The model under review builds one solid part; all positions refer to its coordinate system, in mm. Face numbers are marked on the shaded views. Coordinates: 2 decimals unless noted, no trailing zeros. Loops run counter-clockwise (first coordinate to the right, second up) from the corner with the lowest first, then second, coordinate; pieces in that order, holes last. Notation, with made-up numbers: (41.5, 21.25) - (54.5, 21.25) arc R27 cw to (54.5, 44.25) - close; hole circle Ø5 at (5.5, 55). An arc over 180 degrees is marked (long way). One line per item, written item: value. Start each with the question number.
1. We need section B-B, the plane z = -6.5. Give the boundary of the cut face in (x, y), then the cut area to 3 significant figures.
2. We need section C-C, the plane x = 20. Give the boundary of the cut face in (y, z), then the cut area to 3 significant figures.
3. To check wall thickness, follow line 1 (X direction, y = 4.25, z = 16); line 2 (X direction, y = 9.1, z = 20); line 3 (Y direction, x = -10, z = -3). State the ranges of each line that lie inside material, in increasing order.
4. We need section A-A, the plane x = 0. Give the boundary of the cut face in (y, z), then the cut area to 3 significant figures.
5. Insertion check: P1, Ø3.5, axis at x = 16.5, z = -15.5, coming from the -Y side; P2, Ø1.8, axis at x = -16, z = 16, coming from the -Y side; P3, Ø14, axis at x = -2.5, z = -9.5, coming from the +Y side. Each pin has a flat end and moves straight along its axis. Give the tip position at first contact, or say it passes through.
6. We need section D-D, the plane z = 20. Give the boundary of the cut face in (x, y), then the cut area to 3 significant figures.
7. Mouldability with a two-part tool opening along Z and no side actions: class the marked faces 1, 2 and 3 as +Z half, -Z half, draft (parallel to the pull), parting line (faces both ways), or undercut.
from build123d import *

# Parameters (mm, degrees)
SKETCH1_W           = 50
SKETCH1_H           = 50
BOSS_EXTRUDE1_DEPTH = 10
SKETCH2_R           = 23
CUT_EXTRUDE1_DEPTH  = 3
SKETCH3_R           = 1.5
CUT_EXTRUDE2_DEPTH  = 3
SKETCH4_W           = 50
SKETCH4_H           = 4
CUT_EXTRUDE3_DEPTH  = 76
FILLET1_R           = 3
SKETCH5_R           = 1.5
CUT_EXTRUDE4_DEPTH  = 1


with BuildPart() as part:
    # Sketch1 → Boss-Extrude1 (new body)
    with BuildSketch(Plane(origin=(0, 0, 0), x_dir=(1, 0, 0), z_dir=(0, 1, 0))):
        Rectangle(SKETCH1_W, SKETCH1_H)
    extrude(amount=BOSS_EXTRUDE1_DEPTH)

    # Sketch2 → Cut-Extrude1 (cut)
    with BuildSketch(Plane(origin=(0, 10, 0), x_dir=(1, 0, 0), z_dir=(0, 1, 0))):
        with Locations(Location((0, 0, 0), (0, 0, 270))):
            Circle(SKETCH2_R)
    extrude(amount=-CUT_EXTRUDE1_DEPTH, mode=Mode.SUBTRACT)

    # Sketch3 → Cut-Extrude2 (cut)
    with BuildSketch(Plane(origin=(0, 10, 0), x_dir=(1, 0, 0), z_dir=(0, 1, 0))):
        with Locations(Location((20, -20, 0), (0, 0, 270))):
            Circle(SKETCH3_R)
    extrude(amount=-CUT_EXTRUDE2_DEPTH, mode=Mode.SUBTRACT)

    # Sketch4 → Cut-Extrude3 (cut)
    with BuildSketch(Plane.XY.offset(25)):
        with Locations((0, 2)):
            Rectangle(SKETCH4_W, SKETCH4_H)
    extrude(amount=-CUT_EXTRUDE3_DEPTH, mode=Mode.SUBTRACT)

    # Fillet1
    fillet1_edges = [part.edges().sort_by_distance(p)[0] for p in [
        (25, 7, 25),
        (-25, 7, 25),
        (-25, 7, -25),
        (25, 7, -25),
    ]]
    fillet(fillet1_edges, radius=FILLET1_R)

    # Sketch5 → Cut-Extrude4 (cut)
    with BuildSketch(Plane.XZ.offset(-4)):
        with Locations(Location((-16, 16, 0), (0, 0, 270))):
            Circle(SKETCH5_R)
        with Locations(Location((16, 16, 0), (0, 0, 270))):
            Circle(SKETCH5_R)
        with Locations(Location((-16, -16, 0), (0, 0, 270))):
            Circle(SKETCH5_R)
        with Locations(Location((16, -16, 0), (0, 0, 270))):
            Circle(SKETCH5_R)
    extrude(amount=-CUT_EXTRUDE4_DEPTH, mode=Mode.SUBTRACT)


solid = part.part
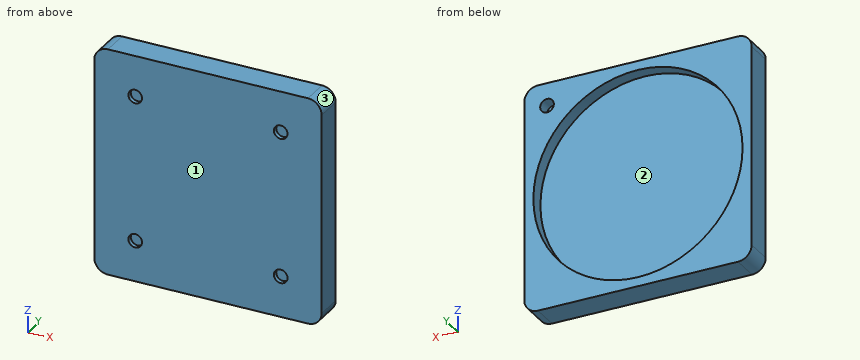
Findings below:
1. outline: (-25, 4) - (25, 4) - (25, 10) - (22.06, 10) - (22.06, 7) - (-22.06, 7) - (-22.06, 10) - (-25, 10) - close
1. area: 168 mm2
2. outline: (4, -25) - (10, -25) - (10, -11.36) - (7, -11.36) - (7, 11.36) - (10, 11.36) - (10, 18.5) - (7, 18.5) - (7, 21.5) - (10, 21.5) - (10, 25) - (4, 25) - close
2. area: 223 mm2
3. line 1: -25 to -17.5, -14.5 to 14.5, 17.5 to 25
3. line 2: -25 to -11.36, 11.36 to 18.5, 21.5 to 25
3. line 3: 4 to 7
4. outline: (4, -25) - (10, -25) - (10, -23) - (7, -23) - (7, 23) - (10, 23) - (10, 25) - (4, 25) - close
4. area: 162 mm2
5. P1: y = 4
5. P2: y = 5
5. P3: y = 7
6. outline: (-25, 4) - (25, 4) - (25, 10) - (21.5, 10) - (21.5, 7) - (18.5, 7) - (18.5, 10) - (11.36, 10) - (11.36, 7) - (-11.36, 7) - (-11.36, 10) - (-25, 10) - close
6. area: 223 mm2
7. face 1: draft
7. face 2: undercut
7. face 3: +Z half
